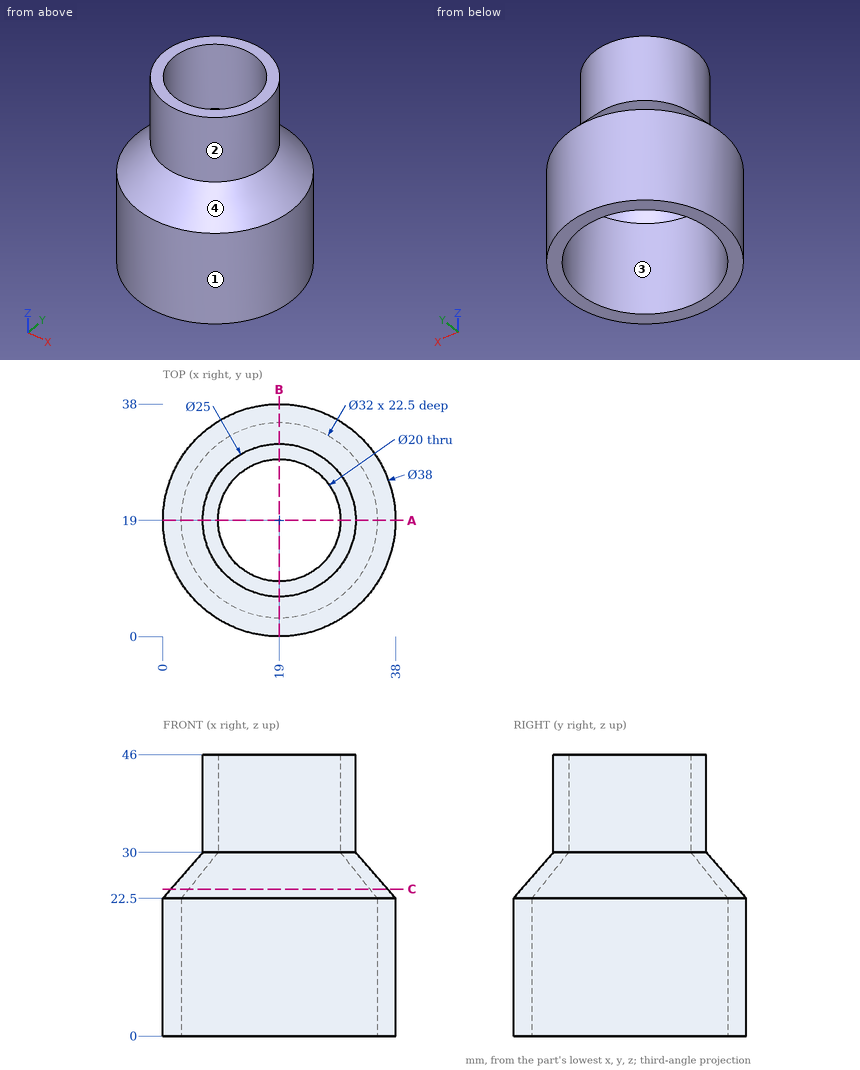
Print and shaded views of the part. All mm, measured from the part's lowest x, y and z. A direction names the side the tool comes from. Give positions to 0.01 mm unless a question says otherwise; leave off trailing zeros. Order: outer loops, then holes, each group sorted by start corner. A loop starts at its lowest first (then second) coordinate and runs counter-clockwise, first axis right, second up. Notation, with made-up numbers: (32.5, -3.75) - (82.5, -3.75) arc R19 ccw to (82.5, 19.25) - close; hole circle Ø1 at (-36, 76.25). An arc over 180 degrees is marked (long way). One line per item, written item: value.
Item 1: Slice it at A-A (y = 19). List the corners of the cut face in (x, z), then the cut area to 3 significant figures.
Response values:
outline: (0, 0) - (3, 0) - (3, 22.5) - (9, 30) - (9, 46) - (6.5, 46) - (6.5, 30) - (0, 22.5) - close; (29, 30) - (35, 22.5) - (35, 0) - (38, 0) - (38, 22.5) - (31.5, 30) - (31.5, 46) - (29, 46) - close
area: 256 mm2
Item 2: Two-plate mould, pull along Y, no slides. Class the marked faces 3 and 4: released by +Y, released by -Y, zero draft, split by the parting line, or undercut.
Response values:
face 3: undercut
face 4: split by the parting line
Item 3: Tool access for the marked faces 1 and 2: list every direction of +Z, -Z, +X, -X, +Y, -Y with a clear straight run to the whole face (end or side of a thin tool).
Response values:
face 1: +Z, -Z
face 2: +Z
Item 4: Pin check, flat tips, straight feed: pin 1 Ø10 at (x, z) = (13, 37) entering from -Y; pin 2 Ø5 at (x, z) = (30.5, 30.5) entering from -Y; pin 3 Ø10 at (x, y) = (15.5, 19.5) entering from -Z; pin 4 Ø12 at (x, z) = (30, 14.5) entering from -Y. Stop position of each tip, or through.
Response values:
pin 1: y = 6.54
pin 2: y = 9.48
pin 3: through
pin 4: y = 0.67
Item 5: Slice it at C-C (z = 24). List the corners of the cut face in (x, y).
Response values:
outline: circle Ø35.4 at (19, 19); hole circle Ø29.6 at (19, 19)
Item 6: Wall check: line 1 (X direction, y = 19, z = 38.5); line 2 (Y direction, x = 19, z = 16). Give the ranges that are in metal, low to high.
Response values:
line 1: 6.5 to 9, 29 to 31.5
line 2: 0 to 3, 35 to 38
